```python
from build123d import *

# Parameters (mm, degrees)
C_CLIP_BODY_DEPTH      = 10
FLANGE_HOLE_1_SKETCH_R = 1.5
FLANGE_HOLE_1_3_DEPTH  = 100
FLANGE_HOLE_2_SKETCH_R = 1.5
FLANGE_HOLE_2_3_DEPTH  = 100
WEB_HOLE_SKETCH_R      = 2.5
WEB_HOLE_5_DEPTH       = 100


with BuildPart() as part:
    # C Clip Profile Sketch → C Clip Body (new body)
    with BuildSketch(Plane.XY):
        with BuildLine():
            Line((0, 0), (0, 28))
            Line((0, 28), (9, 37))
            Line((9, 37), (25, 37))
            Line((25, 37), (25, 32))
            Line((25, 32), (22, 32))
            Line((22, 32), (22, 34))
            Line((22, 34), (14, 34))
            Line((14, 34), (14, 32))
            Line((14, 32), (11.899494937, 32))
            ThreePointArc((11.899494937, 32), (11.134128072, 31.847759065), (10.485281374, 31.414213562))
            Line((10.485281374, 31.414213562), (5.585786438, 26.514718626))
            ThreePointArc((5.585786438, 26.514718626), (5.152240935, 25.865871928), (5, 25.100505063))
            Line((5, 25.100505063), (5, 7))
            ThreePointArc((5, 7), (5.585786438, 5.585786438), (7, 5))
            Line((7, 5), (14, 5))
            Line((14, 5), (14, 3))
            Line((14, 3), (22, 3))
            Line((22, 3), (22, 5))
            Line((22, 5), (25, 5))
            Line((25, 5), (25, 0))
            Line((25, 0), (0, 0))
        make_face()
    extrude(amount=C_CLIP_BODY_DEPTH)

    # Flange Hole 1 Sketch → Flange Hole 1 Ø3 (cut)
    with BuildSketch(Plane(origin=(0, 3, 0), x_dir=(1, 0, 0), z_dir=(0, 1, 0))):
        with Locations(Location((18, -5, 0), (0, 0, 270))):
            Circle(FLANGE_HOLE_1_SKETCH_R)
    extrude(amount=-FLANGE_HOLE_1_3_DEPTH, mode=Mode.SUBTRACT)

    # Flange Hole 2 Sketch → Flange Hole 2 Ø3 (cut)
    with BuildSketch(Plane(origin=(0, 37, 0), x_dir=(1, 0, 0), z_dir=(0, 1, 0))):
        with Locations(Location((18, -5, 0), (0, 0, 270))):
            Circle(FLANGE_HOLE_2_SKETCH_R)
    extrude(amount=-FLANGE_HOLE_2_3_DEPTH, mode=Mode.SUBTRACT)

    # Web Hole Sketch → Web Hole Ø5 (cut)
    with BuildSketch(Plane.ZY):
        with Locations((5, 12)):
            Circle(WEB_HOLE_SKETCH_R)
    extrude(amount=-WEB_HOLE_5_DEPTH, mode=Mode.SUBTRACT)


solid = part.part
```
Could you check a few things on this model? Use its own coordinates, in mm. A direction names the side the tool comes from. Round coordinates to 2 decimals unless told otherwise and drop trailing zeros. Write each loop counter-clockwise with the first axis right and the second up, starting at its lowest first coordinate (ties: lowest second). Pieces come first, ordered by that corner, then holes. Notation, with made-up numbers: M 17,36 L 27,36 A20 cw 27,62 Z; hole C -21,5.5 d5. An arc over 180 degrees is marked long. Write each question's results on one line, items separated by ' | '. Start each with the question number.
1. Imagine slicing it at B-B on x = 18. List the corners of the cut face in (y, z) for me.
2. Thinking about a two-plate mould opening in X: for faces 1 (the face through (11.14, 31.85, 4.93)), 2 (the face through (19.265, 1.521, 5.806)), 3 (the face through (15, 37, 5)), which applies, +X half, -X half, draft (parallel to the pull), parting line (faces both ways), or undercut?
3. I need wall thicknesses on L1, parallel to X at y = 1.05, z = 5; L2, parallel to Y at x = 15.25, z = 6.5; L3, parallel to X at y = 20, z = 2. Which ranges of each line are inside material? Lowest first, please. Write a range as from..to.
4. Imagine slicing it at D-D on x = 2. List the corners of the cut face in (y, z) for me.
5. On a 3-axis mill with a long thin cutter (end or side, diameter ignored), from which of +Z, -Z, +X, -X, +Y, -Y can I reach the whole of each face in a straight line? I mean faces 4 (the face through (25, 3, 5)), 5 (the face through (16, 3, 5)), 6 (the face through (5, 16, 5)). Say none if no direction works.
6. Imagine slicing it at A-A on y = 12. List the corners of the cut face in (x, z) for me.
7. I'm going to push flat-ended pins straight in: pin 1 Ø1 at (y, z) = (33.5, 5.5) entering from -X; pin 2 Ø6 at (y, z) = (28, 2) entering from +X. Where does each tip first touch, or does it pass through?
8. Imagine slicing it at C-C on z = 5. Count the separate pieces of the cut face and the enclosed holes in it, and give its area (3 significant figures).
Result sheet:
1) outline: M 0,0 L 3,0 L 3,3.5 L 0,3.5 Z; M 0,6.5 L 3,6.5 L 3,10 L 0,10 Z; M 34,0 L 37,0 L 37,3.5 L 34,3.5 Z; M 34,6.5 L 37,6.5 L 37,10 L 34,10 Z
2) face 1: +X half | face 2: undercut | face 3: draft
3) L1: x = 0..16.5, 19.5..25 | L2: y = 0..3, 34..37 | L3: x = 0..5
4) outline: M 0,0 L 30,0 L 30,10 L 0,10 Z; hole C 12,5 d5
5) face 4: +Z, -Z, +X, +Y, -Y | face 5: +Z, -Z | face 6: +Z, -Z, +X
6) outline: M 0,0 L 5,0 L 5,2.5 L 0,2.5 Z; M 0,7.5 L 5,7.5 L 5,10 L 0,10 Z
7) pin 1: stops at x = 5 | pin 2: stops at x = 10.07
8) separate pieces: 4 | enclosed holes: 0 | area: 289 mm^2
